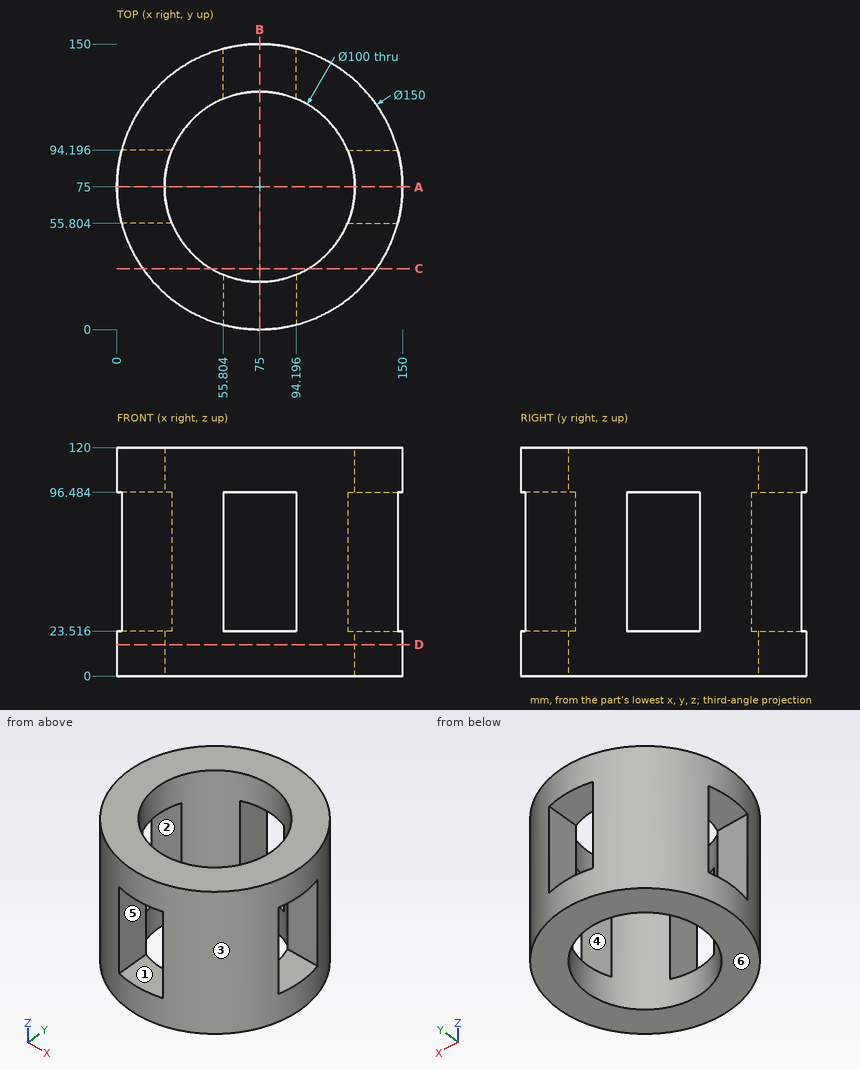
Verification items for this drawing (mm, ordinates from the low corner). A direction names the side the tool comes from. Round coordinates to 2 decimals unless told otherwise and drop trailing zeros. Write each loop counter-clockwise with the first axis right and the second up, starting at its lowest first coordinate (ties: lowest second). Pieces come first, ordered by that corner, then holes. Notation, with made-up numbers: (89.5, 17.5) - (122.5, 17.5) arc R7 ccw to (122.5, 24.5) - close; hole circle Ø10 at (66, 63). An arc over 180 degrees is marked (long way). Answer as a JSON object with one key per item and string values. Group by question number.
Q1. Section check A-A, the plane y = 75. Enter the section's corners in (x, z) (1 decimal), plus the area to 3 significant figures.
Q2. Tool access check on the marked faces 4, 5 and 6. Record the directions out of +Z, -Z, +X, -X, +Y, -Y that give a thin tool (end or side, any length) a straight path to the whole face; none if there is none.
Q3. Go/stop test with flat-tipped pins: pin 1 Ø3 at (x, z) = (25, 72.5) entering from -Y; pin 2 Ø2 at (y, z) = (134.5, 103.5) entering from -X (1 decimal); pin 3 Ø13 at (y, z) = (129, 67.5) entering from -X. Record where each tip stops, or that it passes through.
Q4. Mould release check, pull along Y, two halves, no side actions. Record for the marked faces 1, 2 and 3: released by +Y, released by -Y, zero draft, split by the parting line, or undercut.
Q5. Thickness scan on line 1 (Z direction, x = 16.5, y = 72) (1 decimal); line 2 (X direction, y = 67, z = 7) (1 decimal); line 3 (Y direction, x = 101, z = 101). Record the ranges inside material, lowest first.
Q6. Section check D-D, the plane z = 16.5. Enter the section's corners in (x, y).
Q7. Section check C-C, the plane y = 32. Enter the section's corners in (x, z) (1 decimal).
Found:
{
 "1": {"outline": "(0, 0) - (25, 0) - (25, 23.5) - (0, 23.5) - close; (0, 96.5) - (25, 96.5) - (25, 120) - (0, 120) - close; (125, 0) - (150, 0) - (150, 23.5) - (125, 23.5) - close; (125, 96.5) - (150, 96.5) - (150, 120) - (125, 120) - close", "area": "2,350 mm^2"},
 "2": {"face 4": "+X, -X", "face 5": "+Y, -Y", "face 6": "-Z, +X, -X, +Y, -Y"},
 "3": {"pin 1": "stops at y = 17.79", "pin 2": "stops at x = 28.1", "pin 3": "stops at x = 16.96"},
 "4": {"face 1": "zero draft", "face 2": "undercut", "face 3": "split by the parting line"},
 "5": {"line 1": "z = 0 to 23.5, 96.5 to 120", "line 2": "x = 0.4 to 25.6, 124.4 to 149.6", "line 3": "y = 4.65 to 32.29, 117.71 to 145.35"},
 "6": {"outline": "circle Ø150 at (75, 75); hole circle Ø100 at (75, 75)"},
 "7": {"outline": "(13.6, 0) - (49.5, 0) - (49.5, 120) - (13.6, 120) - close; (100.5, 0) - (136.4, 0) - (136.4, 120) - (100.5, 120) - close"}
}
